Job drawing, mm, ordinate dimensions from the low corner. One solid piece. Round coordinates to 2 decimals unless told otherwise and drop trailing zeros. Order: outer loops, then holes, each group sorted by start corner. A loop starts at its lowest first (then second) coordinate and runs counter-clockwise, first axis right, second up. Notation, with made-up numbers: (42.25, 54.5) -> (71.25, 54.5) arc R17 ccw to (71.25, 63.5) -> close; hole circle Ø1 at (51, -33). An arc over 180 degrees is marked (long way). Return JSON: item names as keys, results as strings. Group by question number.
Q1. Probe line 1 along X through (y, z) = (14.5, 6.5); line 2 along Y through (x, z) = (50, 8.25); line 3 along X through (y, z) = (14, 6.5). List the from-to ranges inside material, lowest first.
Q2. Cut at A-A (x = 30). Write the cut outline in (y, z), then the cut area to 3 significant figures.
Q3. Cut at B-B (y = 37). Write the cut outline in (x, z), then the cut area to 3 significant figures.
Q4. Mould opens along X. For the marked faces 1, 2, 3 and 4 say: +X half, -X half, draft (parallel to the pull), parting line (faces both ways), or undercut.
Q5. Cut at C-C (z = 8.25). Write the cut outline in (x, y), then the cut area to 3 significant figures.
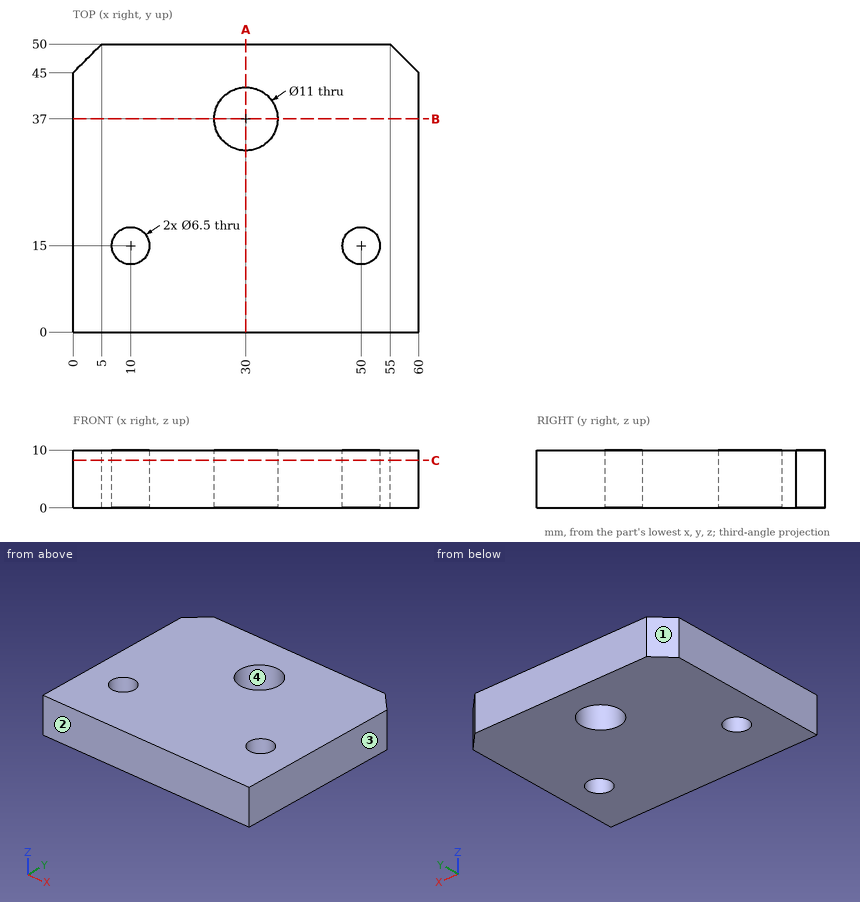
Solution:
{
 "1": {"line 1": "x = 0 to 6.79, 13.21 to 46.79, 53.21 to 60", "line 2": "y = 0 to 11.75, 18.25 to 50", "line 3": "x = 0 to 6.91, 13.09 to 46.91, 53.09 to 60"},
 "2": {"outline": "(0, 0) -> (31.5, 0) -> (31.5, 10) -> (0, 10) -> close; (42.5, 0) -> (50, 0) -> (50, 10) -> (42.5, 10) -> close", "area": "390 mm²"},
 "3": {"outline": "(0, 0) -> (24.5, 0) -> (24.5, 10) -> (0, 10) -> close; (35.5, 0) -> (60, 0) -> (60, 10) -> (35.5, 10) -> close", "area": "490 mm²"},
 "4": {"face 1": "-X half", "face 2": "draft", "face 3": "+X half", "face 4": "undercut"},
 "5": {"outline": "(0, 0) -> (60, 0) -> (60, 45) -> (55, 50) -> (5, 50) -> (0, 45) -> close; hole circle Ø6.5 at (10, 15); hole circle Ø11 at (30, 37); hole circle Ø6.5 at (50, 15)", "area": "2,810 mm²"}
}
